Work out the finished part from the listing and answer in its coordinate system (mm). A direction names the side the tool comes from. Round coordinates to 2 decimals unless told otherwise and drop trailing zeros. Order: outer loops, then holes, each group sorted by start corner. A loop starts at its lowest first (then second) coordinate and runs counter-clockwise, first axis right, second up. Notation, with made-up numbers: M 88,62.5 L 121,62.5 A17 cw 121,77.5 Z; hole C 4.5,-3.5 d7. An arc over 180 degrees is marked long. Return JSON: item names as keys, results as strings.
from build123d import *

# Parameters (mm, degrees)
SKETCH1_W           = 65
SKETCH1_H           = 30
BOSS_EXTRUDE1_DEPTH = 840
SKETCH2_W           = 59
SKETCH2_H           = 24
CUT_EXTRUDE1_DEPTH  = 950
SKETCH5_R           = 3
CUT_EXTRUDE3_DEPTH  = 842.512657385


with BuildPart() as part:
    # Sketch1 → Boss-Extrude1 (new body)
    with BuildSketch(Plane.XY):
        with Locations((-8.040751589, 24.808027615)):
            Rectangle(SKETCH1_W, SKETCH1_H)
    extrude(amount=BOSS_EXTRUDE1_DEPTH)

    # Sketch2 → Cut-Extrude1 (cut)
    with BuildSketch(Plane.XY.offset(840)):
        with Locations((-8.040751589, 24.808027615)):
            Rectangle(SKETCH2_W, SKETCH2_H)
    extrude(amount=-CUT_EXTRUDE1_DEPTH, mode=Mode.SUBTRACT)

    # Sketch5 → Cut-Extrude3 (cut, through all)
    with BuildSketch(Plane(origin=(0, 9.808027615, 0), x_dir=(-1, 0, 0), z_dir=(0, -1, 0))):
        with Locations(Location((8.040751589, -395, 0), (0, 0, 90))):
            Circle(SKETCH5_R)
        with Locations(Location((33.040751589, -420, 0), (0, 0, 90))):
            Circle(SKETCH5_R)
        with Locations(Location((8.040751589, -445, 0), (0, 0, 90))):
            Circle(SKETCH5_R)
        with Locations(Location((-16.959248411, -420, 0), (0, 0, 90))):
            Circle(SKETCH5_R)
    extrude(amount=-CUT_EXTRUDE3_DEPTH, mode=Mode.SUBTRACT)


solid = part.part
Item 1: Which of the six approach directions +Z, -Z, +X, -X, +Y, -Y give full straight-line access (tool end or side, diameter ignored) to faces 1 (the flat face through (-10.6, 12.656, 840)), 2 (the flat face through (-8, 36.808, 426))?
Output:
{"face 1": "+Z, +X, -X, +Y, -Y", "face 2": "+Z, -Z"}
Item 2: The mould has two halves that part along X. Classify faces 3 (the flat face through (-8, 12.808, 426)), 4 (the flat face through (-40.541, 25, 414)), 5 (the flat face through (-8, 9.808, 414)): pulls with the +X half, pulls with the -X half, needs draft (parallel to the pull), parting line crosses it, or undercut.
Output:
{"face 3": "undercut", "face 4": "pulls with the -X half", "face 5": "needs draft"}
Item 3: This flat-tipped pin is pushed along its axis until it touches: pin 1 (8 mm diameter, centred on x = -33.04, z = 420, fed in from -Y). Where does it stop, or does it pass through?
Output:
{"pin 1": "stops at y = 9.81"}
Item 4: Consider line 1 along X through (y, z) = (38.2, 420); line 2 along Z through (x, y) = (-8, 11.5); line 3 along Y through (x, z) = (-8, 307). Determine where each line is inside the solid, lowest interval first. Write a range as [from, to].
Output:
{"line 1": "x = [-40.54, -36.04], [-30.04, 13.96], [19.96, 24.46]", "line 2": "z = [0, 392], [398, 442], [448, 840]", "line 3": "y = [9.81, 12.81], [36.81, 39.81]"}
Item 5: Find section A-A (z = 613). Determine the outline of the cut face in (x, y), plus the area to 3 significant figures.
Output:
{"outline": "M -40.54,9.81 L 24.46,9.81 L 24.46,39.81 L -40.54,39.81 Z; hole M -37.54,12.81 L 21.46,12.81 L 21.46,36.81 L -37.54,36.81 Z", "area": "534 mm^2"}
Item 6: Find section B-B (y = 30.25). Determine the outline of the cut face in (x, z).
Output:
{"outline": "M -40.54,0 L -37.54,0 L -37.54,840 L -40.54,840 Z; M 21.46,0 L 24.46,0 L 24.46,840 L 21.46,840 Z"}
